Can you work these out from the model? Positions are in its coordinate system, mm. Give positions to 0.01 mm unless a question says otherwise; leave off trailing zeros. Order: outer loops, then holes, each group sorted by start corner. A loop starts at its lowest first (then second) coordinate and runs counter-clockwise, first axis right, second up. Notation, with made-up numbers: (16.5, 28.5) - (59.5, 28.5) arc R22 cw to (59.5, 38.5) - close; hole circle Ø6 at (37.5, 55). An arc over 180 degrees is marked (long way). Use one line per item in the form item = value. Start each with the question number.
1) Suppose I cut it at B-B, the plane x = 15. Write out the boundary of the cut face in (y, z), and give its area (3 significant figures).
2) Suppose I cut it at A-A, the plane z = 629. Write out the boundary of the cut face in (x, y), and give its area (3 significant figures).
3) For pin 1 (12 mm diameter, centred on y = 24, z = 323.5, fed in from +X); pin 2 (1 mm diameter, centred on x = 15.5, z = 576, fed in from +Y), each with a flat end and sliding along its axis, tell me the tip position at first contact or that it passes through.
4) Please list where these lines run through material, in increasing order: probe 1 along X at (y, z) = (32.5, 444); probe 2 along X at (y, z) = (3.5, 919).
```python
from build123d import *

# Parameters (mm, degrees)
BOSS_EXTRUDE1_DEPTH = 1020


with BuildPart() as part:
    # Sketch1 → Boss-Extrude1 (new body)
    with BuildSketch(Plane.XY):
        with BuildLine():
            Line((0, 0), (0, 40))
            Line((0, 40), (2.666666667, 40))
            ThreePointArc((2.666666667, 40), (3.609475708, 39.609475708), (4, 38.666666667))
            Line((4, 38.666666667), (4, 9))
            ThreePointArc((4, 9), (5.464466094, 5.464466094), (9, 4))
            Line((9, 4), (38.666666667, 4))
            ThreePointArc((38.666666667, 4), (39.609475708, 3.609475708), (40, 2.666666667))
            Line((40, 2.666666667), (40, 0))
            Line((40, 0), (0, 0))
        make_face()
    extrude(amount=BOSS_EXTRUDE1_DEPTH)


solid = part.part
```
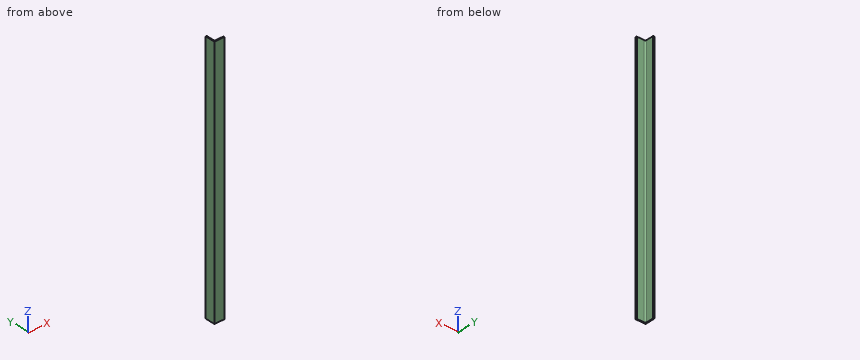
Result sheet:
q1.outline = (0, 0) - (4, 0) - (4, 1020) - (0, 1020) - close
q1.area = 4,080 mm²
q2.outline = (0, 0) - (40, 0) - (40, 2.67) arc R1.33 ccw to (38.67, 4) - (9, 4) arc R5 cw to (4, 9) - (4, 38.67) arc R1.33 ccw to (2.67, 40) - (0, 40) - close
q2.area = 309 mm²
q3.pin_1 = 4
q3.pin_2 = 4
q4.probe_1 = 0 to 4
q4.probe_2 = 0 to 39.71
